Geometry: see drawing. Coordinates: mm, zero at the bounding-box minimum. Coordinates: 2 decimals unless noted, no trailing zeros. Write each loop counter-clockwise with the first axis right and the second up, starting at its lowest first coordinate (ties: lowest second). Pieces come first, ordered by that corner, then holes. Notation, with made-up numbers: (53.25, 60) - (61.25, 60) arc R10 cw to (61.25, 68) - close; hole circle Ø7 at (45.25, 7.5). An arc over 180 degrees is marked (long way). One line per question, with ' | ' between items. Start each with the question number.
1) Section query A-A on x = 55. Return loops of the section in (y, z).
2) Section query C-C on y = 6. Return loops of the section in (x, z), and give its area (3 significant figures).
3) Line query: line 1 (X direction, y = 4.25, z = 55); line 2 (Z direction, x = 47, y = 8.75); line 3 (Z direction, x = 95.5, y = 3.75). Output: solid intervals per line, ascending.
4) Section query B-B on z = 55. Return loops of the section in (x, y), and give its area (4 significant figures).
5) First-contact query: P1, Ø4, axis at x = 43.5, y = 9, coming from the +Z side; P2, Ø6, axis at x = 46.5, y = 6, coming from the +Z side; P3, Ø4, axis at x = 58, y = 2, coming from the +Z side. Flat tips, straight axial feed; report the tip coordinate or a pass-through.
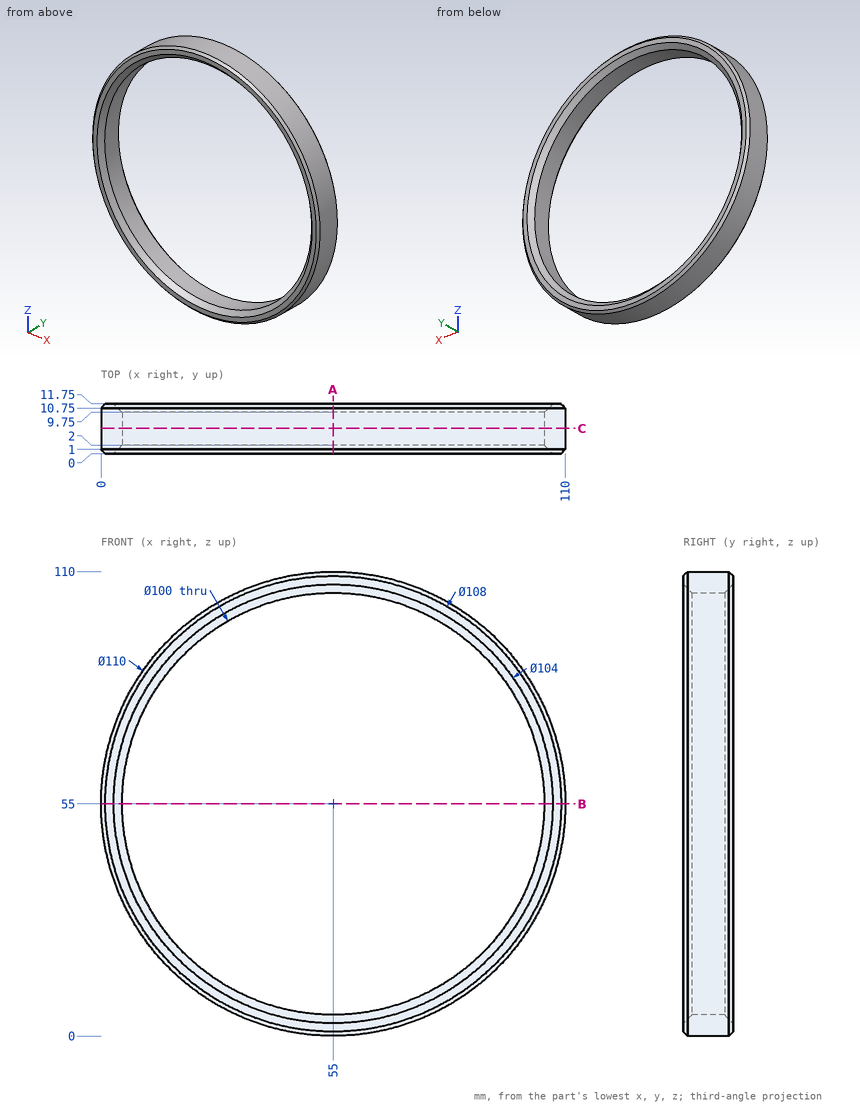
Answer key:
1) outline: (0, 1) - (1, 0) - (10.75, 0) - (11.75, 1) - (11.75, 3) - (9.75, 5) - (2, 5) - (0, 3) - close; (0, 107) - (2, 105) - (9.75, 105) - (11.75, 107) - (11.75, 109) - (10.75, 110) - (1, 110) - (0, 109) - close
2) outline: circle Ø110 at (55, 55); hole circle Ø100 at (55, 55) | area: 1,650 mm²
3) line 1: 0 to 5, 105 to 110 | line 2: 0.58 to 5.64, 104.36 to 109.42 | line 3: 17.79 to 25.68, 84.32 to 92.21
4) outline: (0, 1) - (1, 0) - (3, 0) - (5, 2) - (5, 9.75) - (3, 11.75) - (1, 11.75) - (0, 10.75) - close; (105, 2) - (107, 0) - (109, 0) - (110, 1) - (110, 10.75) - (109, 11.75) - (107, 11.75) - (105, 9.75) - close | area: 107.5 mm²
5) P1: z = 109.17 | P2: z = 109.72 | P3: z = 109.99
